```python
from build123d import *

# Parameters (mm, degrees)
SKETCH1_R  = 0.85
BODY_DEPTH = 1
FILLET1_R  = 0.2
FILLET2_R  = 0.5


with BuildPart() as part:
    # Sketch1 → Body (new body)
    with BuildSketch(Plane.XY):
        with BuildLine():
            Line((-1, -7.327151675), (-1, -10.95227248))
            ThreePointArc((-1, -10.95227248), (-2.900753364, -10.591364126), (-4.703022713, -9.887841997))
            Line((-4.703022713, -9.887841997), (-5.296977287, -6.519358222))
            ThreePointArc((-5.296977287, -6.519358222), (0, 8.4), (5.296977287, -6.519358222))
            Line((5.296977287, -6.519358222), (4.703022713, -9.887841997))
            ThreePointArc((4.703022713, -9.887841997), (2.900753364, -10.591364126), (1, -10.95227248))
            Line((1, -10.95227248), (1, -7.327151675))
            ThreePointArc((1, -7.327151675), (0, 6.4), (-1, -7.327151675))
        make_face()
        with Locations(Location((3, -8.666394553, 0), (0, 0, 180))):
            Circle(SKETCH1_R, mode=Mode.SUBTRACT)
        with Locations((-3, -8.666394553)):
            Circle(SKETCH1_R, mode=Mode.SUBTRACT)
    extrude(amount=-BODY_DEPTH)

    # Fillet1
    fillet1_edges = [part.edges().sort_by_distance(p)[0] for p in [
        (-4.703022713, -9.887841997, -0.5),
        (4.703022713, -9.887841997, -0.5),
    ]]
    fillet(fillet1_edges, radius=FILLET1_R)

    # Fillet2
    fillet2_edges = [part.edges().sort_by_distance(p)[0] for p in [
        (-5.296977287, -6.519358222, -0.5),
        (5.296977287, -6.519358222, -0.5),
    ]]
    fillet(fillet2_edges, radius=FILLET2_R)


solid = part.part
```
Could you check a few things on this model? Use its own coordinates, in mm. A direction names the side the tool comes from. Round coordinates to 2 decimals unless told otherwise and drop trailing zeros. Loops run counter-clockwise (first coordinate to the right, second up) from the corner with the lowest first, then second, coordinate; pieces in that order, holes last. Notation, with made-up numbers: M -5.5,-14.75 L 21.5,-14.75 A20 ccw 21.5,8.25 Z; hole C 9.5,-12.5 d1. An arc over 180 degrees is marked long. Answer as CSV lines item,"result".
1) We'd pull the mould along X, two halves only. Please class faces 1 (the cylindrical face through (2.877, -10.598, -0.493)), 2 (the flat face through (1, -9.2, -0.5)), 3 (the cylindrical face through (-0.287, 8.395, -0.493)): released by +X, released by -X, zero draft, split by the parting line, or undercut.
From the geometry:
face 1,"released by +X"
face 2,"undercut"
face 3,"split by the parting line"
2) For pin 1 Ø0.5 at (y, z) = (-9, -0.5) entering from -X, with a flat end and sliding along its axis, tell me the tip position at first contact or that it passes through.
From the geometry:
pin 1,"x = -4.9"
3) Which directions (+Z, -Z, +X, -X, +Y, -Y) give clear straight access to the entire face, cutting with the end or side of a thin tool? Please do faces 4 (the flat face through (-4.99, -8.27, -0.49)), 5 (the flat face through (-1, -9.1, -0.5)).
From the geometry:
face 4,"+Z, -Z, -X, -Y"
face 5,"+Z, -Z, -Y"
4) Imagine slicing it at C-C on y = -7. List the corners of the cut face in (x, z) for me.
From the geometry:
outline,"M -5.21,-1 L -2.32,-1 L -2.32,0 L -5.21,0 Z; M 2.32,-1 L 5.21,-1 L 5.21,0 L 2.32,0 Z"
5) If I drill on probe 1 along X at (y, z) = (-8, -0.9); probe 2 along Y at (x, z) = (-3.75, -0.9); probe 3 along Y at (x, z) = (-2.75, -0.75), over which ranges is the centre line in solid material (lowest first)?
From the geometry:
probe 1,"-5.04 to -3.53, -2.47 to -1, 1 to 2.47, 3.53 to 5.04"
probe 2,"-10.31 to -9.07, -8.27 to -6.29, 5.29 to 7.52"
probe 3,"-10.63 to -9.48, -7.85 to -6.83, 5.83 to 7.94"
6) Imagine slicing it at A-A on y = -9. List the corners of the cut face in (x, z) for me, and give its area (3 significant figures).
From the geometry:
outline,"M -4.86,-1 L -3.78,-1 L -3.78,0 L -4.86,0 Z; M -2.22,-1 L -1,-1 L -1,0 L -2.22,0 Z; M 1,-1 L 2.22,-1 L 2.22,0 L 1,0 Z; M 3.78,-1 L 4.86,-1 L 4.86,0 L 3.78,0 Z"
area,"4.59 mm^2"
7) Imagine slicing it at B-B on x = -3.5. List the corners of the cut face in (y, z) for me, and give its area (3 significant figures).
From the geometry:
outline,"M -10.4,-1 L -9.35,-1 L -9.35,0 L -10.4,0 Z; M -7.98,-1 L -6.45,-1 L -6.45,0 L -7.98,0 Z; M 5.45,-1 L 7.64,-1 L 7.64,0 L 5.45,0 Z"
area,"4.77 mm^2"
8) Imagine slicing it at D-D on z = -0.15. List the corners of the cut face in (x, y) for me, and give its area (3 significant figures).
From the geometry:
outline,"M -5.43,-6.41 A0.5 cw -5.27,-6.7 L -4.72,-9.79 A0.2 ccw -4.61,-9.93 A10.5 ccw -1,-10.95 L -1,-7.33 A6.9 cw long 1,-7.33 L 1,-10.95 A10.5 ccw 4.61,-9.93 A0.2 ccw 4.72,-9.79 L 5.27,-6.7 A0.5 cw 5.43,-6.41 A8.4 ccw long Z; hole C -3,-8.67 d1.7; hole C 3,-8.67 d1.7"
area,"87.5 mm^2"
